from build123d import *

# Parameters (mm, degrees)
EXTRUDE_1_DEPTH = 50
SHELL_1_T       = -3


with BuildPart() as part:
    # 草图1 → 凸台-拉伸1 (new body)
    with BuildSketch(Plane.XY):
        Polygon((0, 0), (0, 50), (-80, 50), (-80, 30), align=None)
    extrude(amount=EXTRUDE_1_DEPTH)

    # 抽壳1
    shell_1_openings = [part.faces().sort_by_distance(p)[0] for p in [
        (-80, 40, 25),
        (0, 25, 25),
        (-40, 15, 25),
    ]]
    offset(amount=SHELL_1_T, openings=shell_1_openings, kind=Kind.INTERSECTION)


solid = part.part
Check sheet for the modelled part. Datum: model origin and axes. Units: mm. A direction names the side the tool comes from. Round coordinates to 2 decimals unless told otherwise and drop trailing zeros. Loops run counter-clockwise (first coordinate to the right, second up) from the corner with the lowest first, then second, coordinate; pieces in that order, holes last. Notation, with made-up numbers: M 25.25,39 L 56.25,39 A26 ccw 56.25,64 Z; hole C -31.75,78.25 d1. An arc over 180 degrees is marked long. One line per item, written item: value.
(1) Thickness scan on line 1 (Z direction, x = -62, y = 27.5); line 2 (Y direction, x = -50, z = 34). Record the ranges inside material, lowest first.
Computed values:
line 1: z = 0 to 3, 47 to 50
line 2: y = 47 to 50
(2) Sectioned sample at B-B, the plane x = -10. Record the cut outline in (y, z), then the cut area to 4 significant figures.
Computed values:
outline: M 3.75,0 L 50,0 L 50,50 L 3.75,50 L 3.75,47 L 47,47 L 47,3 L 3.75,3 Z
area: 409.5 mm^2
(3) Sectioned sample at D-D, the plane z = 39.5. Record the cut outline in (x, y), then the cut area to 3 significant figures.
Computed values:
outline: M -80,47 L 0,47 L 0,50 L -80,50 Z
area: 240 mm^2
(4) Sectioned sample at C-C, the plane y = 36. Record the cut outline in (x, z).
Computed values:
outline: M -80,0 L 0,0 L 0,3 L -80,3 Z; M -80,47 L 0,47 L 0,50 L -80,50 Z
(5) Sectioned sample at A-A, the plane y = 9. Record the cut outline in (x, z).
Computed values:
outline: M -24,0 L 0,0 L 0,3 L -24,3 Z; M -24,47 L 0,47 L 0,50 L -24,50 Z
(6) Depth check by flat-ended pin: pin 1 Ø22 at (x, z) = (-27.5, 35) entering from -Y. Enter the tip coordinate at first touch or a pass-through.
Computed values:
pin 1: stops at y = 47
(7) Release check for a two-part mould opening along Z. For faces 3 (the face through (-32, 29, 47)), 4 (the face through (-40.56, 15.21, 48.48)), 5 (the face through (-39, 47, 25)), 6 (the face through (-32, 31, 0)) record: +Z half, -Z half, draft (parallel to the pull), parting line (faces both ways), or undercut.
Computed values:
face 3: undercut
face 4: draft
face 5: undercut
face 6: -Z half
(8) Access from +Z, -Z, +X, -X, +Y, -Y to the whole of each face (thin tool, end or side, straight path). Record for faces 1 (the face through (-39, 50, 25)), 2 (the face through (-32, 29, 3)).
Computed values:
face 1: +Z, -Z, +X, -X, +Y
face 2: +X, -X, -Y
